```python
from build123d import *

# Parameters (mm, degrees)
SKETCH_1_W             = 42
SKETCH_1_H             = 72
EXTRUDE_1_DEPTH        = 5
HOLE_WIZARD_M4_2_D     = 3.3
HOLE_WIZARD_M4_2_DEPTH = 12
HOLE_WIZARD_M4_2_TIP   = 0.991420021
SKETCH_6_R             = 16
CUT_EXTRUDE_1_DEPTH    = 43.860237983
CHAMFER_2_SIZE         = 10
FILLET_1_R             = 5
SKETCH_15_W            = 77.686914385
SKETCH_15_H            = 52.90814048
CUT_EXTRUDE_3_DEPTH    = 31
FILLET_2_R             = 5
HOLE_WIZARD_M4_1_D     = 3.3


with BuildPart() as part:
    # 草图1 → 凸台-拉伸1 (new, symmetric)
    with BuildSketch(Plane(origin=(0, 0, 0), x_dir=(1, 0, 0), z_dir=(0, 1, 0))):
        Rectangle(SKETCH_1_W, SKETCH_1_H)
    extrude(amount=EXTRUDE_1_DEPTH, both=True)

    # M4 螺纹孔2
    with Locations(Plane(origin=(0, 0, -36), x_dir=(-1, 0, 0), z_dir=(0, 0, -1))):
        with Locations((-15, 0), (15, 0)):
            Hole(HOLE_WIZARD_M4_2_D / 2, depth=HOLE_WIZARD_M4_2_DEPTH)
            with Locations((0, 0, -(HOLE_WIZARD_M4_2_DEPTH + HOLE_WIZARD_M4_2_TIP / 2))):  # 118° drill point
                Cone(0, HOLE_WIZARD_M4_2_D / 2, HOLE_WIZARD_M4_2_TIP, mode=Mode.SUBTRACT)

    # 草图6 → 切除-拉伸1 (cut, through all)
    with BuildSketch(Plane(origin=(0, 5, 0), x_dir=(1, 0, 0), z_dir=(0, 1, 0))):
        with Locations(Location((0, 1, 0), (0, 0, 270))):
            Circle(SKETCH_6_R)
    extrude(amount=-CUT_EXTRUDE_1_DEPTH, mode=Mode.SUBTRACT)

    # 倒角2
    chamfer_2_edges = [part.edges().sort_by_distance(p)[0] for p in [
        (21, 0, 36),
        (-21, 0, 36),
    ]]
    chamfer(chamfer_2_edges, length=CHAMFER_2_SIZE)

    # 圆角1
    fillet_1_edges = [part.edges().sort_by_distance(p)[0] for p in [
        (11, 0, 36),
        (-11, 0, 36),
        (-21, 0, 26),
        (21, 0, 26),
    ]]
    fillet(fillet_1_edges, radius=FILLET_1_R)

    # 草图15 → 切除-拉伸3 (cut)
    with BuildSketch(Plane(origin=(0, 5, 0), x_dir=(1, 0, 0), z_dir=(0, 1, 0))):
        with Locations((6.233739535, -45.45407024)):
            Rectangle(SKETCH_15_W, SKETCH_15_H)
    extrude(amount=-CUT_EXTRUDE_3_DEPTH, mode=Mode.SUBTRACT)

    # 圆角2
    fillet_2_edges = [part.edges().sort_by_distance(p)[0] for p in [
        (21, 0, 19),
        (-21, 0, 19),
    ]]
    fillet(fillet_2_edges, radius=FILLET_2_R)

    # M4 螺纹孔1 (through all)
    with Locations(Plane(origin=(0, 5, 0), x_dir=(1, 0, 0), z_dir=(0, 1, 0))):
        with Locations((-16.265, 17.265), (16.265, 17.265), (-16.265, -15.265), (16.265, -15.265)):
            Hole(HOLE_WIZARD_M4_1_D / 2)


solid = part.part
```
Input: part model. Units: mm. Frame: model coordinates. A direction names the side the tool comes from. Coordinates: 2 decimals unless noted, no trailing zeros. Write each loop counter-clockwise with the first axis right and the second up, starting at its lowest first coordinate (ties: lowest second). Pieces come first, ordered by that corner, then holes. Notation, with made-up numbers: M -22.75,34.5 L 0.25,34.5 A15 ccw 0.25,53.5 Z; hole C -17,-30 d4. An arc over 180 degrees is marked long. Use one line per item in the form item = value.
Q1. Section B-B (z = -1). Return loops of the section in (x, y), plus the area to 3 significant figures.
Answer below:
outline = M -21,-5 L -16,-5 L -16,5 L -21,5 Z; M 16,-5 L 21,-5 L 21,5 L 16,5 Z
area = 100 mm²
Q2. Draft query along Z for faces 3 (the face through (0, 0, -36)), 4 (the face through (0, -5, -21)), 5 (the face through (-17.026, -0.07, -15.801)). Return one class per face: released by +Z, released by -Z, zero draft, split by the parting line, or undercut.
Answer below:
face_3 = released by -Z
face_4 = zero draft
face_5 = undercut
Q3. Material intervals for probe 1 along X at (y, z) = (0, -32.5); probe 2 along X at (y, z) = (3.5, -18.5); probe 3 along X at (y, z) = (0.75, -1), sorted ascending. Write a range as from..to.
Answer below:
probe_1 = -21..-16.65, -13.35..13.35, 16.65..21
probe_2 = -21..-17.36, -15.17..15.17, 17.36..21
probe_3 = -21..-16, 16..21
Q4. Section A-A (x = -10). Return loops of the section in (y, z).
Answer below:
outline = M -5,-36 L 5,-36 L 5,-13.49 L -5,-13.49 Z; M -5,11.49 L 5,11.49 L 5,19 L -5,19 Z
Q5. Set-up query: faces 1 (the face through (16.623, -0.07, -15.654)), 2 (the face through (16.574, 0.496, -29.916)). Return all of +Z, -Z, +X, -X, +Y, -Y with unobstructed straight access to the full face (end or side cutting, diameter ignored); none if empty.
Answer below:
face_1 = +Y, -Y
face_2 = -Z
Q6. Section D-D (y = 0.75). Count the separate pieces of the cut face and the enclosed holes in it, plus the area to 3 significant figures.
Answer below:
separate_pieces = 1
enclosed_holes = 5
area = 1,390 mm²
Q7. Section C-C (y = 3.5). Return loops of the section in (x, z) (3 decimals).
Answer below:
outline = M -21,-36 L 21,-36 L 21,14 A5 ccw 16,19 L -16,19 A5 ccw -21,14 Z; hole C -16.265,-17.265 d3.3; hole C -16.265,15.265 d3.3; hole C 0,-1 d32; hole C 16.265,-17.265 d3.3; hole C 16.265,15.265 d3.3
